from build123d import *

# Parameters (mm, degrees)
SKETCH_1_R      = 2
SKETCH_1_R_2    = 16
SKETCH_1_R_3    = 3.91899873
SKETCH_1_R_4    = 3
EXTRUDE_1_DEPTH = 15


with BuildPart() as part:
    # 草图1 → 凸台-拉伸1 (new body)
    with BuildSketch(Plane.XY):
        with BuildLine():
            Line((-14, 112), (-6, 0))
            ThreePointArc((-6, 0), (0, -6), (6, 0))
            add(Edge.make_bspline(
                [(6, 0), (1.588652615, 45.680929706), (5.604102499, 63.643200211), (28.004797731, 96.13093391)],
                knots=[0, 0, 0, 0, 0.788155359, 0.788155359, 0.788155359, 0.788155359], degree=3))
            ThreePointArc((28.004797731, 96.13093391), (50.113637924, 112.900750568), (77, 119.767416406))
            ThreePointArc((77, 119.767416406), (157.787149523, 154.485384951), (196.379869136, 233.494896157))
            ThreePointArc((196.379869136, 233.494896157), (200.439238403, 236.311917913), (202, 241))
            Line((202, 241), (202, 246))
            ThreePointArc((202, 246), (194.5, 253.5), (187, 246))
            ThreePointArc((187, 246), (154.781745931, 168.218254069), (77, 136))
            Line((77, 136), (10, 136))
            ThreePointArc((10, 136), (-6.970562748, 128.970562748), (-14, 112))
        make_face()
        Circle(SKETCH_1_R, mode=Mode.SUBTRACT)
        with Locations((10, 112)):
            Circle(SKETCH_1_R_2, mode=Mode.SUBTRACT)
        with Locations((194.5, 246)):
            Circle(SKETCH_1_R_3, mode=Mode.SUBTRACT)
        with Locations((0, 22)):
            Circle(SKETCH_1_R_4, mode=Mode.SUBTRACT)
    extrude(amount=EXTRUDE_1_DEPTH)


solid = part.part
For this review, take the finished solid that the model builds, in its own axes (mm). A direction names the side the tool comes from. Round coordinates to 2 decimals unless told otherwise and drop trailing zeros. Order: outer loops, then holes, each group sorted by start corner. A loop starts at its lowest first (then second) coordinate and runs counter-clockwise, first axis right, second up. Notation, with made-up numbers: M 32,26.25 L 46,26.25 A13 cw 46,44.25 Z; hole C 48,9 d6. An arc over 180 degrees is marked long. Use a Markdown table: item, result. Add a question column.
Item 1: Tool access review of faces 1 (the cylindrical face through (200.4, 236.26, 7.4)), 2 (the flat face through (44, 136, 7)): name each direction out of +Z, -Z, +X, -X, +Y, -Y from which nothing blocks a thin tool from reaching the whole face with its end or side.
Item 2: To check wall thickness, follow line 1 along Y through (x, z) = (0, 8); line 2 along Y through (x, z) = (24, 7.5); line 3 along X through (y, z) = (100.5, 6.5). State the ranges of each line that lie inside material, in increasing order.
Item 3: Add section A-A, the plane z = 12.25. State how many separate pieces and enclosed holes the cut face has, then the cut area to 3 significant figures.
Item 4: Add section C-C, the plane y = 180.5. Give the boundary of the cut face in (x, z), then the cut area to 3 significant figures.
Item 5: Add section B-B, the plane x = 90.5. Give the boundary of the cut face in (y, z), then the cut area to 3 significant figures.
Item 6: Mouldability with a two-part tool opening along Y and no side actions: class faces 3 (the cylindrical face through (49.76, 112.73, 7.4)), 4 (the cylindrical face through (193.65, 242.174, 7.395)), 5 (the cylindrical face through (155.632, 169.078, 7.395)), 6 (the cylindrical face through (18.6, 125.49, 7.4)) as released by +Y, released by -Y, zero draft, split by the parting line, or undercut.
Item 7: Insertion check: pin 1 (6.5 mm diameter, centred on x = 194.5, y = 246, fed in from -Z); pin 2 (1.5 mm diameter, centred on x = 130, z = 4.5, fed in from -Y); pin 3 (6 mm diameter, centred on x = 94, z = 3, fed in from +Y); pin 4 (6 mm diameter, centred on y = 162.5, z = 3, fed in from -X). Each pin has a flat end and moves straight along its axis. Give the tip position at first contact, or say it passes through.
Geometry results:
| question | item | result |
|---|---|---|
| 1 | face 1 | +Z, -Z, +X, -Y |
| 1 | face 2 | +Z, -Z, -X, +Y |
| 2 | line 1 | y = -6 to -2, 2 to 19, 25 to 99.51, 124.49 to 133.82 |
| 2 | line 2 | y = 90.17 to 104.25, 119.75 to 136 |
| 2 | line 3 | x = -13.18 to -1.12, 21.12 to 32.21 |
| 3 | separate pieces | 1 |
| 3 | enclosed holes | 4 |
| 3 | area | 6,110 mm² |
| 4 | outline | M 165.37,0 L 178.7,0 L 178.7,15 L 165.37,15 Z |
| 4 | area | 200 mm² |
| 5 | outline | M 121.18,0 L 136.83,0 L 136.83,15 L 121.18,15 Z |
| 5 | area | 235 mm² |
| 6 | face 3 | released by -Y |
| 6 | face 4 | undercut |
| 6 | face 5 | released by +Y |
| 6 | face 6 | undercut |
| 7 | pin 1 | passes through |
| 7 | pin 2 | stops at y = 134.03 |
| 7 | pin 3 | stops at y = 137.83 |
| 7 | pin 4 | stops at x = 144.95 |
